Read the model definition and answer for the solid it produces. Units are mm, in the model's axes. A direction names the side the tool comes from. Coordinates: 2 decimals unless noted, no trailing zeros. Loops run counter-clockwise (first coordinate to the right, second up) from the corner with the lowest first, then second, coordinate; pieces in that order, holes last. Notation, with made-up numbers: (-24, 51.25) -> (-10, 51.25) arc R24 cw to (-10, 82.25) -> close; hole circle Ø11 at (-20.5, 76.5). An arc over 180 degrees is marked (long way). Answer as a JSON object with one key per item and string values. Group by question number.
Q1. The part is cut by section D-D on y = 15.5. Write down the section's boundary in (x, z).
Q2. For faces 4 (the cylindrical face through (65, 5, 0)), 5 (the flat face through (-15, 4, 28)), determine the directions among +Z, -Z, +X, -X, +Y, -Y from which every point of the face is accessible in a straight line to the end or side of a thin tool.
Q3. The part is cut by section C-C on z = -12. Write down the section's boundary in (x, y).
Q4. Determine the mould class of faces 1 (the flat face through (30, 0, -9)), 2 (the flat face through (39.733, 4.93, -22.525)), 3 (the cylindrical face through (33.71, 12.11, -4.43)) for opening direction Z: released by +Z, released by -Z, zero draft, split by the parting line, or undercut.
Q5. The part is cut by section B-B on x = -55.5. Write down the section's boundary in (y, z).
Q6. The part is cut by section A-A on z = 0. Write down the section's boundary in (x, y), and give its area (3 significant figures).
Q7. Straight lines are drawn through the part: line 1 along X through (y, z) = (11, 0); line 2 along Z through (x, y) = (26, 6.25); line 3 along X through (y, z) = (14, -22.5). For each, find the intervals that lie inside material, in ascending order. Write a range as [from, to].
Q8. Each of these flat-tipped pins is pushed along its axis until it touches: P1, Ø13, axis at x = 46.5, z = -2, coming from the +Y side; P2, Ø10, axis at x = -15.5, y = 13.5, coming from the +Z side; P3, Ø5, axis at y = 10.5, z = 9, coming from the +X side; P4, Ø13, axis at x = -33, z = 5.5, coming from the +Y side. Where does it stop, or does it pass through?
from build123d import *
from build123d.topology import SkipClean

# Parameters (mm, degrees)
SKETCH_1_R          = 6
EXTRUDE_1_DEPTH     = 10
SKETCH_2_R          = 40
EXTRUDE_2_DEPTH     = 10
SKETCH_3_R          = 34
CUT_EXTRUDE_1_DEPTH = 16
SKETCH_4_R          = 31
CUT_EXTRUDE_2_DEPTH = 16


with BuildPart() as part:
    # 草图1 → 凸台-拉伸1 (new body)
    with BuildSketch(Plane(origin=(0, 0, 0), x_dir=(1, 0, 0), z_dir=(0, 1, 0))):
        with BuildLine():
            Line((-59.047619048, 10.64794275), (-20.952380952, 34.0734168))
            ThreePointArc((-20.952380952, 34.0734168), (0, 40), (20.952380952, 34.0734168))
            Line((20.952380952, 34.0734168), (59.047619048, 10.64794275))
            ThreePointArc((59.047619048, 10.64794275), (65, 0), (59.047619048, -10.64794275))
            Line((59.047619048, -10.64794275), (20.952380952, -34.0734168))
            ThreePointArc((20.952380952, -34.0734168), (0, -40), (-20.952380952, -34.0734168))
            Line((-20.952380952, -34.0734168), (-59.047619048, -10.64794275))
            ThreePointArc((-59.047619048, -10.64794275), (-65, 0), (-59.047619048, 10.64794275))
        make_face()
        with Locations(Location((52.5, 0, 0), (0, 0, 270))):
            Circle(SKETCH_1_R, mode=Mode.SUBTRACT)
        with Locations(Location((-52.5, 0, 0), (0, 0, 270))):
            Circle(SKETCH_1_R, mode=Mode.SUBTRACT)
    extrude(amount=EXTRUDE_1_DEPTH)

    # 草图2 → 凸台-拉伸2 (add)
    with SkipClean():  # the faces are left unmerged after this step: merging them gives an invalid solid
        with BuildSketch(Plane(origin=(0, 10, 0), x_dir=(1, 0, 0), z_dir=(0, 1, 0))):
            with Locations(Location((0, 0, 0), (0, 0, 121.588135505))):
                Circle(SKETCH_2_R)
        extrude(amount=EXTRUDE_2_DEPTH)

    # 草图3 → 切除-拉伸1 (cut)
    with SkipClean():  # the faces are left unmerged after this step: merging them gives an invalid solid
        with BuildSketch(Plane(origin=(0, 20, 0), x_dir=(1, 0, 0), z_dir=(0, 1, 0))):
            with Locations(Location((0, 0, 0), (0, 0, 270))):
                Circle(SKETCH_3_R)
        extrude(amount=-CUT_EXTRUDE_1_DEPTH, mode=Mode.SUBTRACT)

    # 草图4 → 切除-拉伸2 (cut)
    with SkipClean():  # the faces are left unmerged after this step: merging them gives an invalid solid
        with BuildSketch(Plane(origin=(0, 4, 0), x_dir=(1, 0, 0), z_dir=(0, 1, 0))):
            with Locations(Location((0, 0, 0), (0, 0, 270))):
                Circle(SKETCH_4_R)
        extrude(amount=-CUT_EXTRUDE_2_DEPTH, mode=Mode.SUBTRACT)


solid = part.part
Final values:
{
 "1": {"outline": "circle Ø80 at (0, 0); hole circle Ø68 at (0, 0)"},
 "2": {"face 4": "+X, +Y, -Y", "face 5": "+Y"},
 "3": {"outline": "(-56.85, 0) -> (-28.58, 0) -> (-28.58, 4) -> (-31.81, 4) -> (-31.81, 20) -> (-38.16, 20) -> (-38.16, 10) -> (-56.85, 10) -> close; (28.58, 0) -> (56.85, 0) -> (56.85, 10) -> (38.16, 10) -> (38.16, 20) -> (31.81, 20) -> (31.81, 4) -> (28.58, 4) -> close"},
 "4": {"face 1": "zero draft", "face 2": "released by -Z", "face 3": "undercut"},
 "5": {"outline": "(0, -12.83) -> (10, -12.83) -> (10, -5.2) -> (0, -5.2) -> close; (0, 5.2) -> (10, 5.2) -> (10, 12.83) -> (0, 12.83) -> close"},
 "6": {"outline": "(-65, 0) -> (-58.5, 0) -> (-58.5, 10) -> (-65, 10) -> close; (-46.5, 0) -> (-31, 0) -> (-31, 4) -> (-34, 4) -> (-34, 20) -> (-40, 20) -> (-40, 10) -> (-46.5, 10) -> close; (31, 0) -> (46.5, 0) -> (46.5, 10) -> (40, 10) -> (40, 20) -> (34, 20) -> (34, 4) -> (31, 4) -> close; (58.5, 0) -> (65, 0) -> (65, 10) -> (58.5, 10) -> close", "area": "524 mm2"},
 "7": {"line 1": "x = [-40, -34], [34, 40]", "line 2": "z = [-30.97, -21.91], [21.91, 30.97]", "line 3": "x = [-33.07, -25.49], [25.49, 33.07]"},
 "8": {"P1": "stops at y = 10", "P2": "stops at z = 38.6", "P3": "stops at x = 63.15", "P4": "stops at y = 20"}
}
